Check sheet for the drawn part. Datum: minimum x, y, z corner. Units: mm. A direction names the side the tool comes from. Round coordinates to 2 decimals unless told otherwise and drop trailing zeros. Order: outer loops, then holes, each group sorted by start corner. A loop starts at its lowest first (then second) coordinate and runs counter-clockwise, first axis right, second up. Notation, with made-up numbers: (33.25, 82.5) -> (56.25, 82.5) arc R22 ccw to (56.25, 90.5) -> close; hole circle Ø2 at (35.25, -20). An arc over 180 degrees is marked (long way). Use CSV: the item, a comma, the result in double quotes.
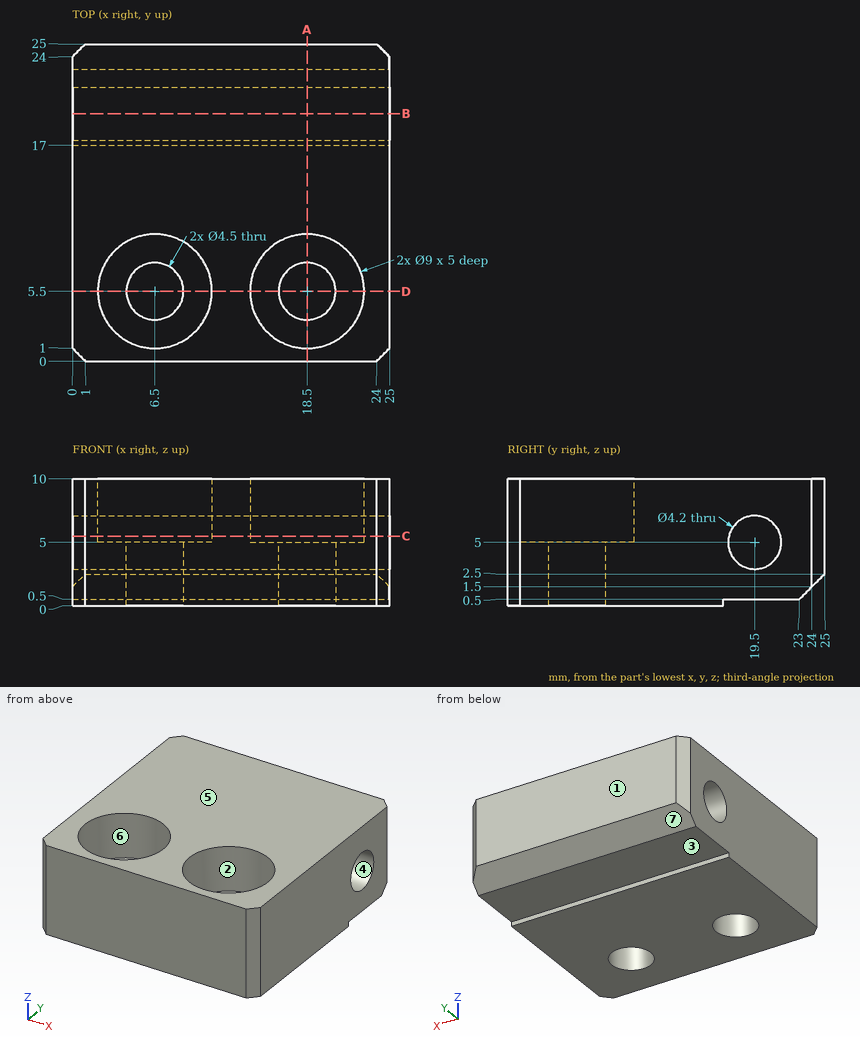
Q1. Sectioned sample at D-D, the plane y = 5.5. Enter the section's corners in (x, z).
Result sheet:
outline,"(0, 0) -> (4.25, 0) -> (4.25, 5) -> (2, 5) -> (2, 10) -> (0, 10) -> close; (8.75, 0) -> (16.25, 0) -> (16.25, 5) -> (14, 5) -> (14, 10) -> (11, 10) -> (11, 5) -> (8.75, 5) -> close; (20.75, 0) -> (25, 0) -> (25, 10) -> (23, 10) -> (23, 5) -> (20.75, 5) -> close"
Q2. Mould release check, pull along Z, two halves, no side actions. Record for the marked faces 4, 5, 6 and 7: pulls with the +Z half, pulls with the -Z half, needs draft (parallel to the pull), parting line crosses it, or undercut.
Result sheet:
face 4,"undercut"
face 5,"pulls with the +Z half"
face 6,"needs draft"
face 7,"pulls with the -Z half"
Q3. Sectioned sample at A-A, the plane x = 18.5. Enter the section's corners in (y, z), then the cut area to 3 significant figures.
Result sheet:
outline,"(0, 0) -> (3.25, 0) -> (3.25, 5) -> (1, 5) -> (1, 10) -> (0, 10) -> close; (7.75, 0) -> (17, 0) -> (17, 0.5) -> (23, 0.5) -> (25, 2.5) -> (25, 10) -> (10, 10) -> (10, 5) -> (7.75, 5) -> close; hole circle Ø4.2 at (19.5, 5)"
area,"163 mm^2"
Q4. Go/stop test with flat-tipped pins: pin 1 (6 mm diameter, centred on x = 18.5, y = 5.5, fed in from +Z); pin 2 (1.8 mm diameter, centred on x = 11, y = 21, fed in from -Z). Record where each tip stops, or that it passes through.
Result sheet:
pin 1,"stops at z = 5"
pin 2,"stops at z = 0.5"
Q5. Scan lines: L1, parallel to Z at x = 19.5, y = 19.5; L2, parallel to Y at x = 6.5, z = 8.2; L3, parallel to X at y = 9.5, z = 8.25. Record each from-to range of solid material in increasing order.
Result sheet:
L1,"z = 0.5 to 2.9, 7.1 to 10"
L2,"y = 0 to 1, 10 to 25"
L3,"x = 0 to 4.44, 8.56 to 16.44, 20.56 to 25"
Q6. Sectioned sample at B-B, the plane y = 19.5. Enter the section's corners in (x, z).
Result sheet:
outline,"(0, 0.5) -> (25, 0.5) -> (25, 2.9) -> (0, 2.9) -> close; (0, 7.1) -> (25, 7.1) -> (25, 10) -> (0, 10) -> close"
Q7. Sectioned sample at C-C, the plane z = 5.5. Enter the section's corners in (x, y).
Result sheet:
outline,"(0, 1) -> (1, 0) -> (24, 0) -> (25, 1) -> (25, 17.46) -> (0, 17.46) -> close; (0, 21.54) -> (25, 21.54) -> (25, 24) -> (24, 25) -> (1, 25) -> (0, 24) -> close; hole circle Ø9 at (6.5, 5.5); hole circle Ø9 at (18.5, 5.5)"
Q8. Access from +Z, -Z, +X, -X, +Y, -Y to the whole of each face (thin tool, end or side, straight path). Record for the marked faces 1, 2 and 3.
Result sheet:
face 1,"+Z, -Z, +X, -X, +Y"
face 2,"+Z"
face 3,"-Z, +X, -X, +Y"
